The drawing under review shows one solid part. Ordinate dimensions are in mm from its lowest x, y, z. Coordinates: 2 decimals unless noted, no trailing zeros. Order: outer loops, then holes, each group sorted by start corner. A loop starts at its lowest first (then second) coordinate and runs counter-clockwise, first axis right, second up.
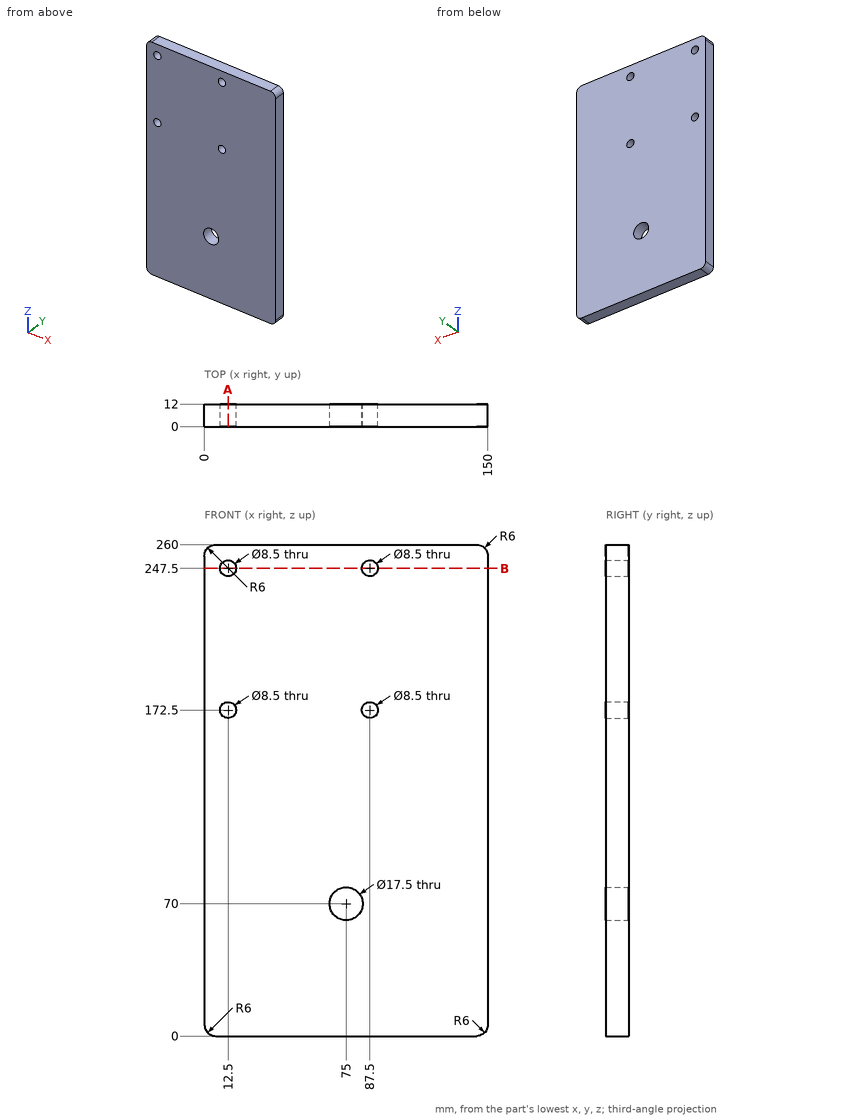
(1) For pin 1 Ø5 at (x, z) = (87.5, 247.5) entering from +Y, flat-tipped, find the tip position at first contact; note if it passes through.
A:
pin 1: passes through
(2) Wall thickness on probe 1 along Z at (x, y) = (87.5, 4); probe 2 along X at (y, z) = (4.25, 172.5); probe 3 along X at (y, z) = (7.75, 70): over which ranges is each line inside the solid? List them lowest first.
A:
probe 1: z = 0 to 168.25, 176.75 to 243.25, 251.75 to 260
probe 2: x = 0 to 8.25, 16.75 to 83.25, 91.75 to 150
probe 3: x = 0 to 66.25, 83.75 to 150
(3) We need section A-A, the plane x = 12.5. Write out the cut boundary in (y, z), and give its area (3 significant figures).
A:
outline: (0, 0) - (12, 0) - (12, 168.25) - (0, 168.25) - close; (0, 176.75) - (12, 176.75) - (12, 243.25) - (0, 243.25) - close; (0, 251.75) - (12, 251.75) - (12, 260) - (0, 260) - close
area: 2,920 mm2
(4) We need section B-B, the plane z = 247.5. Write out the cut boundary in (x, y).
A:
outline: (0, 0) - (8.25, 0) - (8.25, 12) - (0, 12) - close; (16.75, 0) - (83.25, 0) - (83.25, 12) - (16.75, 12) - close; (91.75, 0) - (150, 0) - (150, 12) - (91.75, 12) - close
